Geometry check sheet. Reference: drawing and pictorial views, mm from the part's lowest x, y, z. A direction names the side the tool comes from. Give positions to 0.01 mm unless a question says otherwise; leave off trailing zeros. Write each loop counter-clockwise with the first axis right and the second up, starting at its lowest first coordinate (ties: lowest second). Pieces come first, ordered by that corner, then holes. Notation, with made-up numbers: M 24.5,12.25 L 78.5,12.25 A10 cw 78.5,20.25 Z; hole C 51,41 d11. An arc over 180 degrees is marked long. Write item = value, one per line. Start each with the question number.
1) Go/stop test with flat-tipped pins: pin 1 (7.5 mm diameter, centred on x = 40, z = 15, fed in from +Y); pin 2 (13.5 mm diameter, centred on x = 10, z = 15, fed in from +Y). Record where each tip stops, or that it passes through.
2) Cross-section at B-B, the plane z = 5.5. Record the cut outline in (x, y).
3) Scan lines: line 1 along X through (y, z) = (5, 13); line 2 along Y through (x, z) = (25, 7.5); line 3 along X through (y, z) = (13.5, 14). Record each from-to range of solid material in increasing order. Write a range as [from, to].
4) Cross-section at A-A, the plane x = 25. Record the cut outline in (y, z).
5) Mould release check, pull along Z, two halves, no side actions. Record for the marked faces 3, 4 and 5: released by +Z, released by -Z, zero draft, split by the parting line, or undercut.
6) Cross-section at C-C, the plane x = 45.5. Record the cut outline in (y, z), plus the area to 4 significant figures.
7) Cross-section at D-D, the plane y = 51.5. Record the cut outline in (x, z), plus the area to 3 significant figures.
8) Access from +Z, -Z, +X, -X, +Y, -Y to the whole of each face (thin tool, end or side, straight path). Record for the marked faces 1 and 2.
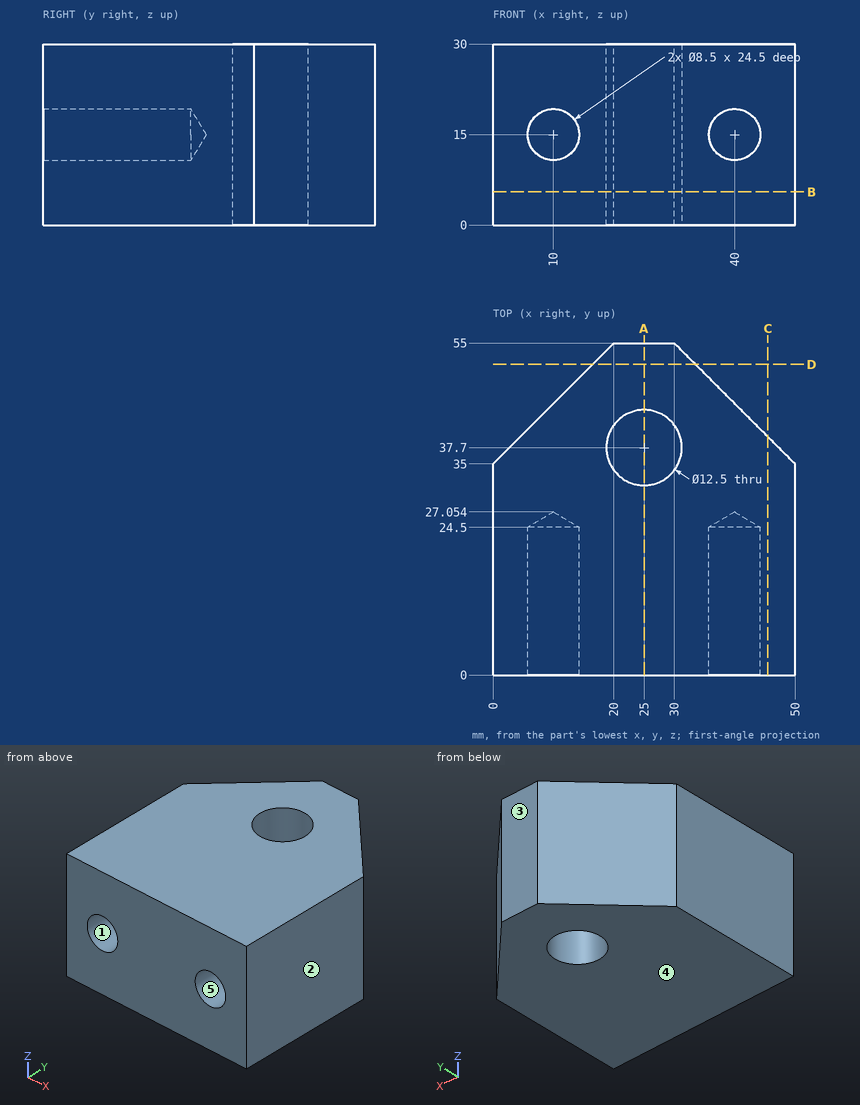
Reply:
q1.pin_1 = 48.75
q1.pin_2 = 51.75
q2.outline = M 0,0 L 50,0 L 50,35 L 30,55 L 20,55 L 0,35 Z; hole C 25,37.7 d12.5
q3.line_1 = [0, 6.25], [13.75, 36.25], [43.75, 50]
q3.line_2 = [0, 31.45], [43.95, 55]
q3.line_3 = [0, 5.87], [14.13, 35.87], [44.13, 50]
q4.outline = M 0,0 L 31.45,0 L 31.45,30 L 0,30 Z; M 43.95,0 L 55,0 L 55,30 L 43.95,30 Z
q5.face_3 = zero draft
q5.face_4 = released by -Z
q5.face_5 = undercut
q6.outline = M 0,0 L 39.5,0 L 39.5,30 L 0,30 Z
q6.area = 1,185 mm2
q7.outline = M 16.5,0 L 33.5,0 L 33.5,30 L 16.5,30 Z
q7.area = 510 mm2
q8.face_1 = -Y
q8.face_2 = +Z, -Z, +X, +Y, -Y
